```python
from build123d import *

# Parameters (mm, degrees)
SKETCH_1_R               = 32
EXTRUDE_1_DEPTH          = 31
CUT_EXTRUDE_1_DEPTH      = 55.854352608
PATTERN_CIRCULAR_1_COUNT = 30
CUT_EXTRUDE_2_DEPTH      = 55.792153984
SKETCH_5_OUTSIDE_W       = 85.106
SKETCH_5_OUTSIDE_H       = 84.892
SKETCH_5_OUTSIDE_R       = 27
CUT_EXTRUDE_3_DEPTH      = 42


with BuildPart() as part:
    # 草图1 → 凸台-拉伸1 (new body)
    with BuildSketch(Plane.XY):
        Circle(SKETCH_1_R)
    extrude(amount=EXTRUDE_1_DEPTH)

    # 草图2 → 切除-拉伸1 (cut, through all)
    with BuildSketch(Plane.XY):
        with BuildLine():
            ThreePointArc((0.291117258, 27.498459061), (0, 27.5), (-0.291117258, 27.498459061))
            add(Edge.make_bspline(
                [(-0.291117258, 27.498459061), (-1.016461379, 27.62595034), (-1.020609493, 28.094265272), (-1.11796964, 28.57715803), (-1.139901483, 28.676258475), (-1.166494173, 28.785849819), (-1.198135434, 28.905795984), (-1.235261247, 29.035929815), (-1.278286716, 29.176077028), (-1.327627025, 29.326048954), (-1.383690587, 29.485644922), (-1.446880683, 29.65465171), (-1.517594534, 29.8328439), (-1.596223153, 30.019983966), (-1.683150964, 30.215822454), (-1.778755503, 30.42009815), (-1.883407094, 30.632538255), (-1.99746854, 30.852858572), (-2.121294814, 31.0807637), (-2.255232758, 31.315947232), (-2.399620786, 31.558091968), (-2.554788592, 31.806870128), (-2.721056861, 32.061943577), (-2.89873699, 32.322964055), (-3.088130814, 32.589573415), (-3.289530328, 32.861403867), (-3.503217435, 33.138078232), (-3.729463678, 33.419210196), (-3.968529992, 33.70440458), (-4.220666464, 33.993257607), (-4.486112085, 34.285357181), (-4.765094529, 34.580283169), (-5.057829915, 34.877607694), (-5.364522622, 35.176895427), (-5.685364966, 35.47770389), (-6.137847732, 35.885241657), (-6.490689237, 36.184143062), (-6.732623663, 36.381116246)],
                knots=[0, 0, 0, 0, 0.115323882, 0.12341257, 0.132512303, 0.142623081, 0.153744905, 0.165877774, 0.179021689, 0.193176649, 0.208342655, 0.224519706, 0.241707802, 0.259906945, 0.279117132, 0.299338365, 0.320570644, 0.342813968, 0.366068337, 0.390333752, 0.415610213, 0.441897719, 0.46919627, 0.497505867, 0.52682651, 0.557158198, 0.588500931, 0.62085471, 0.654219534, 0.688595404, 0.723982319, 0.76038028, 0.797789286, 0.836209338, 0.875640435, 0.916082578, 1, 1, 1, 1], degree=3))
            ThreePointArc((-6.732623663, 36.381116246), (0, 36.998835667), (6.732623663, 36.381116246))
            add(Edge.make_bspline(
                [(0.291117258, 27.498459061), (1.016461379, 27.62595034), (1.020609493, 28.094265272), (1.11796964, 28.57715803), (1.139901483, 28.676258475), (1.166494173, 28.785849819), (1.198135434, 28.905795984), (1.235261247, 29.035929815), (1.278286716, 29.176077028), (1.327627025, 29.326048954), (1.383690587, 29.485644922), (1.446880683, 29.65465171), (1.517594534, 29.8328439), (1.596223153, 30.019983966), (1.683150964, 30.215822454), (1.778755503, 30.42009815), (1.883407094, 30.632538255), (1.99746854, 30.852858572), (2.121294814, 31.0807637), (2.255232758, 31.315947232), (2.399620786, 31.558091968), (2.554788592, 31.806870128), (2.721056861, 32.061943577), (2.89873699, 32.322964055), (3.088130814, 32.589573415), (3.289530328, 32.861403867), (3.503217435, 33.138078232), (3.729463678, 33.419210196), (3.968529992, 33.70440458), (4.220666464, 33.993257607), (4.486112085, 34.285357181), (4.765094529, 34.580283169), (5.057829915, 34.877607694), (5.364522622, 35.176895427), (5.685364966, 35.47770389), (6.137847732, 35.885241657), (6.490689237, 36.184143062), (6.732623663, 36.381116246)],
                knots=[0, 0, 0, 0, 0.115323882, 0.12341257, 0.132512303, 0.142623081, 0.153744905, 0.165877774, 0.179021689, 0.193176649, 0.208342655, 0.224519706, 0.241707802, 0.259906945, 0.279117132, 0.299338365, 0.320570644, 0.342813968, 0.366068337, 0.390333752, 0.415610213, 0.441897719, 0.46919627, 0.497505867, 0.52682651, 0.557158198, 0.588500931, 0.62085471, 0.654219534, 0.688595404, 0.723982319, 0.76038028, 0.797789286, 0.836209338, 0.875640435, 0.916082578, 1, 1, 1, 1], degree=3))
        make_face()
    cut_extrude_1 = extrude(amount=CUT_EXTRUDE_1_DEPTH, mode=Mode.SUBTRACT)

    # 阵列(圆周)1: 切除-拉伸1 ×30 about axis
    pattern_circular_1_axis = Axis((0, 0, 31), (0, 0, -1))
    for i in range(1, PATTERN_CIRCULAR_1_COUNT):
        add(cut_extrude_1.rotate(pattern_circular_1_axis, i * 360 / PATTERN_CIRCULAR_1_COUNT), mode=Mode.SUBTRACT)

    # 草图4 → 切除-拉伸2 (cut, through all)
    with BuildSketch(Plane.XY.offset(31)):
        with BuildLine():
            Line((5, 16.770509831), (5, 20.070509831))
            Line((5, 20.070509831), (-5, 20.070509831))
            Line((-5, 20.070509831), (-5, 16.770509831))
            ThreePointArc((-5, 16.770509831), (0, -17.5), (5, 16.770509831))
        make_face()
    extrude(amount=-CUT_EXTRUDE_2_DEPTH, mode=Mode.SUBTRACT)

    # 草图5 outside → 切除-拉伸3 (cut)
    with BuildSketch(Plane.XY):
        Rectangle(SKETCH_5_OUTSIDE_W, SKETCH_5_OUTSIDE_H)
        Circle(SKETCH_5_OUTSIDE_R, mode=Mode.SUBTRACT)
    extrude(amount=CUT_EXTRUDE_3_DEPTH, mode=Mode.SUBTRACT)


solid = part.part
```
Input: part model. Units: mm. Frame: model coordinates. A direction names the side the tool comes from. Round coordinates to 2 decimals unless told otherwise and drop trailing zeros. Write each loop counter-clockwise with the first axis right and the second up, starting at its lowest first coordinate (ties: lowest second). Pieces come first, ordered by that corner, then holes. Notation, with made-up numbers: (-23.5, 79) -> (12.5, 79) arc R26 cw to (12.5, 103) -> close; hole circle Ø7 at (-7.5, 12.5). An arc over 180 degrees is marked (long way). Answer as CSV lines item,"result".
1. Contact query for flat-ended pins moving along their axis: P1, Ø10, axis at x = -11.5, z = 16.5, coming from the +Y side; P2, Ø5, axis at x = 2, z = 5, coming from the -Y side; P3, Ø2, axis at y = 9, z = 22.5, coming from the -X side; P4, Ø3, axis at x = 15.5, y = 3.5, coming from the +Z side. Output: stop coordinate, or through.
Geometry says:
P1,"stops at y = 26.21"
P2,"stops at y = -27"
P3,"stops at x = -25.79"
P4,"passes through"
2. Section D-D (x = -22.5). Return the cut outline in (y, z).
Geometry says:
outline,"(-14.92, 0) -> (14.92, 0) -> (14.92, 31) -> (-14.92, 31) -> close"
3. Section A-A (y = 0). Return the cut outline in (x, z), plus the area to 3 significant figures.
Geometry says:
outline,"(-27, 0) -> (-17.5, 0) -> (-17.5, 31) -> (-27, 31) -> close; (17.5, 0) -> (27, 0) -> (27, 31) -> (17.5, 31) -> close"
area,"589 mm^2"
4. Section C-C (x = 15.5). Return the cut outline in (y, z), plus the area to 3 significant figures.
Geometry says:
outline,"(-22.11, 0) -> (-8.12, 0) -> (-8.12, 31) -> (-22.11, 31) -> close; (8.12, 0) -> (22.11, 0) -> (22.11, 31) -> (8.12, 31) -> close"
area,"867 mm^2"
5. Mould query, pull axis X, two halves, no side actions, for faces 3 (the cylindrical face through (-5.85, -26.36, 15.28)), 4 (the flat face through (0, 20.071, 16)), 5 (the flat face through (5, 18, 16)), 6 (the flat face through (0, -18, 31)). Classes: +X half, -X half, draft (parallel to the pull), parting line (faces both ways), or undercut.
Geometry says:
face 3,"parting line"
face 4,"undercut"
face 5,"undercut"
face 6,"draft"
6. Ray query, L1, parallel to X at y = 0, z = 29.5; L2, parallel to Y at x = 0, z = 14.5; L3, parallel to Y at x = -1.5, z = 22.5. Return the intervals inside material, ascending. Write a range as [from, to].
Geometry says:
L1,"x = [-27, -17.5], [17.5, 27]"
L2,"y = [-27, -17.5], [20.07, 27]"
L3,"y = [-26.96, -17.44], [20.07, 26.96]"
7. Section B-B (z = 4). Return the cut outline in (x, y), plus the area to 3 significant figures.
Geometry says:
outline,"circle Ø54 at (0, 0); hole (-5, 16.77) arc R17.5 ccw (long way) to (5, 16.77) -> (5, 20.07) -> (-5, 20.07) -> close"
area,"1,300 mm^2"
8. Reachability of faces 1 (the flat face through (0, -18, 0)), 2 (the flat face through (-5, 18, 16)) from +Z, -Z, +X, -X, +Y, -Y: full face, straight path, thin tool, end or side. Return the list, or none.
Geometry says:
face 1,"-Z, +X, -X, +Y, -Y"
face 2,"+Z, -Z"
